from build123d import *

# Parameters (mm, degrees)
SKETCH_1_W                   = 50
SKETCH_1_H                   = 65
EXTRUDE_1_DEPTH              = 5
CHAMFER_1_SIZE               = 10
HOLE_WIZARD_M5_1_D           = 4.2
HOLE_WIZARD_M5_1_DEPTH       = 12.4
HOLE_WIZARD_M5_1_TIP         = 1.2618073
HOLE_WIZARD_M3_1_D           = 3.4
HOLE_WIZARD_M3_1_CBORE_D     = 6.5
HOLE_WIZARD_M3_1_CBORE_DEPTH = 3.4
HOLE_WIZARD_M5_2_D           = 4.2
HOLE_WIZARD_M5_2_DEPTH       = 12.4
HOLE_WIZARD_M5_2_TIP         = 1.2618073


with BuildPart() as part:
    # 草图1 → 凸台-拉伸1 (new, symmetric)
    with BuildSketch(Plane(origin=(0, 0, 0), x_dir=(1, 0, 0), z_dir=(0, 1, 0))):
        Rectangle(SKETCH_1_W, SKETCH_1_H)
    extrude(amount=EXTRUDE_1_DEPTH, both=True)

    # 倒角1
    chamfer_1_edges = [part.edges().sort_by_distance(p)[0] for p in [
        (25, 0, -32.5),
    ]]
    chamfer(chamfer_1_edges, length=CHAMFER_1_SIZE)

    # M5 螺纹孔1
    with Locations(Plane.ZY.offset(25)):
        with Locations((-12.5, 0), (12.5, 0)):
            Hole(HOLE_WIZARD_M5_1_D / 2, depth=HOLE_WIZARD_M5_1_DEPTH)
            with Locations((0, 0, -(HOLE_WIZARD_M5_1_DEPTH + HOLE_WIZARD_M5_1_TIP / 2))):  # 118° drill point
                Cone(0, HOLE_WIZARD_M5_1_D / 2, HOLE_WIZARD_M5_1_TIP, mode=Mode.SUBTRACT)

    # M3 六角凹头螺钉的柱形沉头孔1 (through all)
    with Locations(Plane(origin=(0, -5, 0), x_dir=(-1, 0, 0), z_dir=(0, -1, 0))):
        with Locations((-7, 27.5), (10.960512242, 9.539487758)):
            CounterBoreHole(HOLE_WIZARD_M3_1_D / 2, HOLE_WIZARD_M3_1_CBORE_D / 2, HOLE_WIZARD_M3_1_CBORE_DEPTH)

    # M5 螺纹孔2
    with Locations(Plane.XY.offset(32.5)):
        with Locations((-15, 0), (5, 0)):
            Hole(HOLE_WIZARD_M5_2_D / 2, depth=HOLE_WIZARD_M5_2_DEPTH)
            with Locations((0, 0, -(HOLE_WIZARD_M5_2_DEPTH + HOLE_WIZARD_M5_2_TIP / 2))):  # 118° drill point
                Cone(0, HOLE_WIZARD_M5_2_D / 2, HOLE_WIZARD_M5_2_TIP, mode=Mode.SUBTRACT)


solid = part.part
Can you work these out from the model? Positions are in its coordinate system, mm. A direction names the side the tool comes from. Give positions to 0.01 mm unless a question says otherwise; leave off trailing zeros. Order: outer loops, then holes, each group sorted by start corner. A loop starts at its lowest first (then second) coordinate and runs counter-clockwise, first axis right, second up. Notation, with made-up numbers: (-36, 49.5) - (7, 49.5) arc R17 ccw to (7, 73.5) - close; hole circle Ø9 at (14.25, 34). An arc over 180 degrees is marked (long way). Write each question's results on one line, items separated by ' | '.
1) Please list where these lines run through material, in increasing order: line 1 along Z through (x, y) = (-22.5, -0.25); line 2 along X through (y, z) = (0, 22.75); line 3 along Z through (x, y) = (7, -2.9). Write a range as [from, to].
Final values:
line 1: z = [-32.5, -14.59], [-10.41, 10.41], [14.59, 32.5] | line 2: x = [-25, -17.1], [-12.9, 2.9], [7.1, 25] | line 3: z = [-32.5, -30.75], [-24.25, 32.5]
2) Suppose I cut it at A-A, the plane z = -27.5. Write out the boundary of the cut face in (x, y), then the cut area to 3 significant figures.
Final values:
outline: (-25, -5) - (3.75, -5) - (3.75, -1.6) - (5.3, -1.6) - (5.3, 5) - (-25, 5) - close; (8.7, -1.6) - (10.25, -1.6) - (10.25, -5) - (20, -5) - (20, 5) - (8.7, 5) - close | area: 405 mm^2
3) I'm going to push flat-ended pins straight in: pin 1 Ø2 at (x, z) = (5.5, -26) entering from -Y; pin 2 Ø3.5 at (y, z) = (0, -12.5) entering from -X. Where does each tip first touch, or does it pass through?
Final values:
pin 1: stops at y = -1.6 | pin 2: stops at x = -12.39
4) Suppose I cut it at B-B, the plane y = -4. Write out the boundary of the cut face in (x, z), then the cut area to 3 significant figures.
Final values:
outline: (-25, -32.5) - (15, -32.5) - (25, -22.5) - (25, 32.5) - (-25, 32.5) - close; hole circle Ø6.5 at (-10.96, -9.54); hole circle Ø6.5 at (7, -27.5) | area: 3,130 mm^2
5) On a 3-axis mill with a long thin cutter (end or side, diameter ignored), from which of +Z, -Z, +X, -X, +Y, -Y can I reach the whole of each face in a straight line? I mean faces 4 (the face through (-12.9, 0.09, 26.21)), 5 (the face through (-10.256, -3.324, -6.367)), 6 (the face through (-18.71, 0.09, 14.6)). Say none if no direction works.
Final values:
face 4: +Z | face 5: -Y | face 6: -X
6) If we mould it in two halves opening along Y, with no side actions, what happens to faces 1 (the face through (4.711, -0.222, 19.057)), 2 (the face through (-12, -1.6, -8)), 3 (the face through (-25, 0, 0))? For each: pulls with the +Y half, pulls with the -Y half, needs draft (parallel to the pull), parting line crosses it, or undercut.
Final values:
face 1: undercut | face 2: pulls with the -Y half | face 3: needs draft
